Source: CAD feature listing. Evaluate the final solid. Frame: model axes, mm. Round coordinates to 2 decimals unless told otherwise and drop trailing zeros. Order: outer loops, then holes, each group sorted by start corner. A loop starts at its lowest first (then second) coordinate and runs counter-clockwise, first axis right, second up. Notation, with made-up numbers: M 34,-13.5 L 40,-13.5 A20 cw 40,3.5 Z; hole C 73.25,-16.75 d8. An arc over 180 degrees is marked long. Use one line per item in the form item = value. Start each with the question number.
Q1. Section B-B (z = -3.5). Return the cut outline in (x, y).
Q2. Section C-C (y = -72.5). Return the cut outline in (x, z).
Q3. Material intervals for probe 1 along Y at (x, z) = (0, 3); probe 2 along X at (y, z) = (74, 6); probe 3 along Y at (x, z) = (4, -5), sorted ascending.
Q4. Section A-A (x = 0). Return the cut outline in (y, z), plus the area to 3 significant figures.
Q5. Section D-D (x = -20). Return the cut outline in (y, z).
Q6. Pull-direction query (Y, two-part tool) for faces 1 (the flat face through (-40, -1, 0)), 2 (the cylindrical face through (3.252, -60.357, -0.245)), 3 (the cylindrical face through (0.6, -110, 0.2)); classes: pulls with the +Y half, pulls with the -Y half, needs draft (parallel to the pull), parting line crosses it, or undercut.
Q7. Contact query for flat-ended pins moving along their axis: pin 1 (12 mm diameter, centred on x = -30.5, z = -11, fed in from -Y); pin 2 (5 mm diameter, centred on x = -13, z = 12.5, fed in from +Y); pin 3 (1 mm diameter, centred on x = 13, z = 3.5, fed in from +Y). Output: stop coordinate, or through.
from build123d import *

# Parameters (mm, degrees)
PLATE_PROFILE_WITH_BORES_R = 15
CROSSHEAD_PLATE_35MM_DEPTH = 17.5


with BuildPart() as part:
    # Plate Profile with Bores → Crosshead Plate 35mm (new, symmetric)
    with BuildSketch(Plane.XY):
        with BuildLine():
            Line((-40, -102.46950766), (-40, 102.46950766))
            ThreePointArc((-40, 102.46950766), (0, 110), (40, 102.46950766))
            Line((40, 102.46950766), (40, -102.46950766))
            ThreePointArc((40, -102.46950766), (0, -110), (-40, -102.46950766))
        make_face()
        with Locations((0, 75)):
            Circle(PLATE_PROFILE_WITH_BORES_R, mode=Mode.SUBTRACT)
        with Locations(Location((0, -75, 0), (0, 0, 180))):
            Circle(PLATE_PROFILE_WITH_BORES_R, mode=Mode.SUBTRACT)
    extrude(amount=CROSSHEAD_PLATE_35MM_DEPTH, both=True)


solid = part.part
Results list:
q1.outline = M -40,-102.47 A110 ccw 40,-102.47 L 40,102.47 A110 ccw -40,102.47 Z; hole C 0,-75 d30; hole C 0,75 d30
q2.outline = M -40,-17.5 L -14.79,-17.5 L -14.79,17.5 L -40,17.5 Z; M 14.79,-17.5 L 40,-17.5 L 40,17.5 L 14.79,17.5 Z
q3.probe_1 = -110 to -90, -60 to 60, 90 to 110
q3.probe_2 = -40 to -14.97, 14.97 to 40
q3.probe_3 = -109.93 to -89.46, -60.54 to 60.54, 89.46 to 109.93
q4.outline = M -110,-17.5 L -90,-17.5 L -90,17.5 L -110,17.5 Z; M -60,-17.5 L 60,-17.5 L 60,17.5 L -60,17.5 Z; M 90,-17.5 L 110,-17.5 L 110,17.5 L 90,17.5 Z
q4.area = 5,600 mm2
q5.outline = M -108.17,-17.5 L 108.17,-17.5 L 108.17,17.5 L -108.17,17.5 Z
q6.face_1 = needs draft
q6.face_2 = undercut
q6.face_3 = pulls with the -Y half
q7.pin_1 = -107.24
q7.pin_2 = 109.5
q7.pin_3 = 109.29
